The figure shows three views and two pictorial views of one solid part (mm, origin at its lowest corner). Answer the questions. A direction names the side the tool comes from. Round coordinates to 2 decimals unless told otherwise and drop trailing zeros. Order: outer loops, then holes, each group sorted by start corner. A loop starts at its lowest first (then second) coordinate and runs counter-clockwise, first axis right, second up. Notation, with made-up numbers: (-38.5, 71) -> (-19.5, 71) arc R22 ccw to (-19.5, 105) -> close; hole circle Ø2 at (-21, 82.5). An arc over 180 degrees is marked (long way). Return JSON: item names as keys, results as strings. Group by question number.
(1) The part is cut by section A-A (y = 7.5). Determine the outline of the cut face in (x, z).
(2) The part is cut by section D-D (z = 4.25). Determine the outline of the cut face in (x, y).
(3) Consider line 1 (Y direction, x = 7.5, z = 9.5); line 2 (X direction, y = 13.5, z = 6.75); line 3 (Z direction, x = 9.75, y = 3.75). Determine where each line is inside the solid, lowest interval first. Write a range as [from, to].
(4) Each of these flat-tipped pins is pushed along its axis until it touches: pin 1 (3.5 mm diameter, centred on x = 7.5, y = 7.5, fed in from +Z); pin 2 (6 mm diameter, centred on y = 8, z = 6.5, fed in from +X); pin 3 (2 mm diameter, centred on y = 12.5, z = 3.5, fed in from +X); pin 4 (4.5 mm diameter, centred on x = 9.5, y = 9.5, fed in from -Z). Where does it stop, or does it pass through?
(5) The part is cut by section C-C (z = 13). Determine the outline of the cut face in (x, y), plus the area to 3 significant figures.
(6) Which of the six approach directions +Z, -Z, +X, -X, +Y, -Y give full straight-line access (tool end or side, diameter ignored) to the marked faces 5 and 6?
(7) Determine the mould class of the marked faces 1, 2, 3 and 4 for opening direction X: +X half, -X half, draft (parallel to the pull), parting line (faces both ways), or undercut.
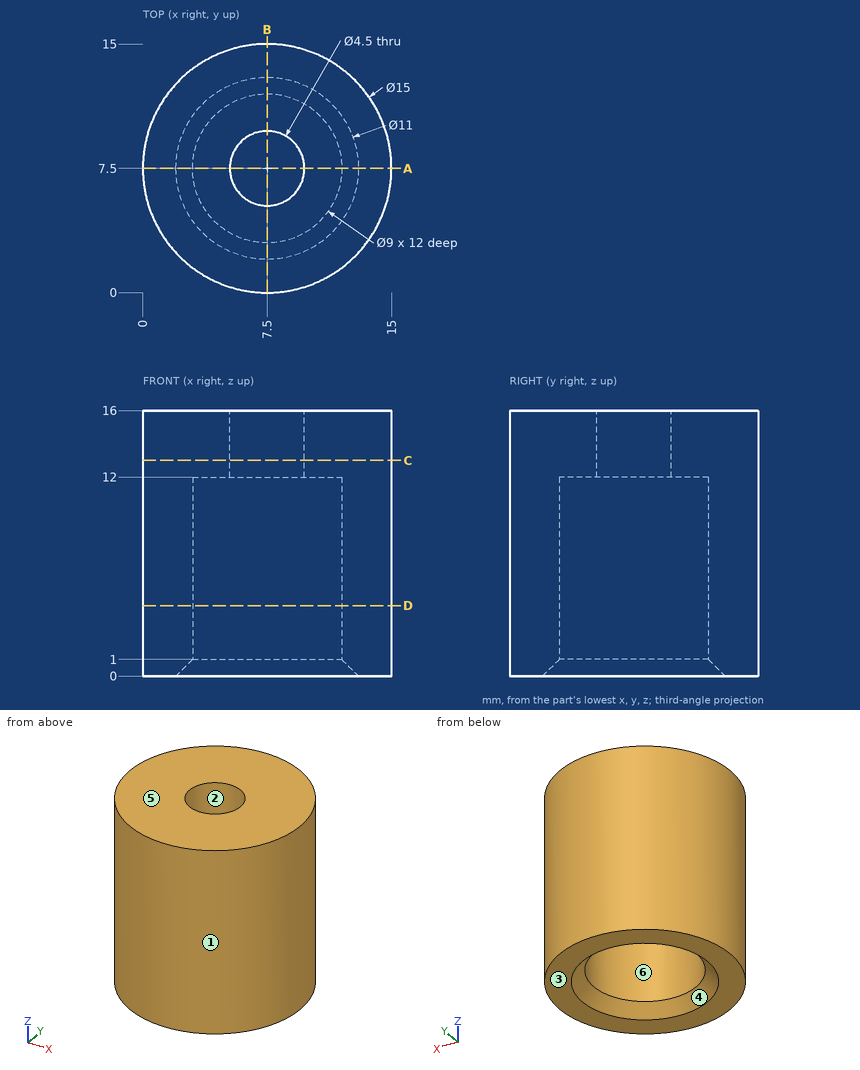
Answer below:
{
 "1": {"outline": "(0, 0) -> (2, 0) -> (3, 1) -> (3, 12) -> (5.25, 12) -> (5.25, 16) -> (0, 16) -> close; (9.75, 12) -> (12, 12) -> (12, 1) -> (13, 0) -> (15, 0) -> (15, 16) -> (9.75, 16) -> close"},
 "2": {"outline": "circle Ø15 at (7.5, 7.5); hole circle Ø9 at (7.5, 7.5)"},
 "3": {"line 1": "y = [0, 3], [12, 15]", "line 2": "x = [3, 12]", "line 3": "z = [12, 16]"},
 "4": {"pin 1": "passes through", "pin 2": "stops at x = 15", "pin 3": "stops at x = 13.84", "pin 4": "stops at z = 0.42"},
 "5": {"outline": "circle Ø15 at (7.5, 7.5); hole circle Ø4.5 at (7.5, 7.5)", "area": "161 mm²"},
 "6": {"face 5": "+Z, +X, -X, +Y, -Y", "face 6": "-Z"},
 "7": {"face 1": "parting line", "face 2": "undercut", "face 3": "draft", "face 4": "undercut"}
}
